```python
from build123d import *

# Parameters (mm, degrees)
SKETCH_1_W                = 1840
SKETCH_1_H                = 120
EXTRUDE_1_DEPTH           = 14
HOLE_WIZARD_1_D           = 6.6
HOLE_WIZARD_1_CBORE_D     = 11
HOLE_WIZARD_1_CBORE_DEPTH = 6.8
HOLE_WIZARD_M5_1_D        = 4.2
PATTERN_LINEAR_1_COUNT    = 27
PATTERN_LINEAR_1_PITCH    = 60
HOLE_WIZARD_12_5_12_5_2_D = 12.5
SKETCH_8_R                = 15
CUT_EXTRUDE_1_DEPTH       = 923.060735527
HOLE_WIZARD_M6_1_D        = 5
PATTERN_LINEAR_2_COUNT    = 4
PATTERN_LINEAR_2_PITCH    = 510
HOLE_WIZARD_8_5_8_5_1_D   = 8.5
SKETCH_13_R               = 42.5
CUT_EXTRUDE_2_DEPTH       = 3


with BuildPart() as part:
    # 草图1 → 凸台-拉伸1 (new body)
    with BuildSketch(Plane(origin=(0, 0, 0), x_dir=(0, 0, -1), z_dir=(1, 0, 0))):
        Rectangle(SKETCH_1_W, SKETCH_1_H)
    extrude(amount=EXTRUDE_1_DEPTH)

    # 打孔尺寸(%根据)内六角圆柱头螺钉的类型1 (through all)
    with Locations(Plane(origin=(0, 0, 0), x_dir=(0, 0, -1), z_dir=(-1, 0, 0))):
        with Locations((-896.162950904, -16.162950904), (-843.837049096, -16.162950904), (-896.162950904, 36.162950904), (-843.837049096, 36.162950904)):
            CounterBoreHole(HOLE_WIZARD_1_D / 2, HOLE_WIZARD_1_CBORE_D / 2, HOLE_WIZARD_1_CBORE_DEPTH)

    # M5 螺纹孔1 (through all)
    with Locations(Plane(origin=(14, 0, 0), x_dir=(0, 0, -1), z_dir=(1, 0, 0))):
        with Locations((-775, 26)):
            hole_wizard_m5_1 = Hole(HOLE_WIZARD_M5_1_D / 2)

    # 阵列(线性)1: M5 螺纹孔1 ×27
    with Locations(*[(0, 0, -i * PATTERN_LINEAR_1_PITCH) for i in range(1, PATTERN_LINEAR_1_COUNT)]):
        add(hole_wizard_m5_1, mode=Mode.SUBTRACT)

    # Ø12.5 (12.5) 直径孔2 (through all)
    with Locations(Plane(origin=(14, 0, 0), x_dir=(0, 0, -1), z_dir=(1, 0, 0))):
        with Locations((845, 25), (895, 25), (845, -25), (895, -25)):
            Hole(HOLE_WIZARD_12_5_12_5_2_D / 2)

    # 草图8 → 切除-拉伸1 (cut, through all)
    with BuildSketch(Plane(origin=(14, 0, 0), x_dir=(0, 0, -1), z_dir=(1, 0, 0))):
        with Locations((-870, -10)):
            Circle(SKETCH_8_R)
    extrude(amount=-CUT_EXTRUDE_1_DEPTH, mode=Mode.SUBTRACT)

    # M6 螺纹孔1 (through all)
    with Locations(Plane.ZY):
        with Locations((780, -40)):
            hole_wizard_m6_1 = Hole(HOLE_WIZARD_M6_1_D / 2)

    # 阵列(线性)2: M6 螺纹孔1 ×4
    with Locations(*[(0, 0, -i * PATTERN_LINEAR_2_PITCH) for i in range(1, PATTERN_LINEAR_2_COUNT)]):
        add(hole_wizard_m6_1, mode=Mode.SUBTRACT)

    # Ø8.5 (8.5) 直径孔1 (through all)
    with Locations(Plane(origin=(14, 0, 0), x_dir=(0, 0, -1), z_dir=(1, 0, 0))):
        with Locations((-910, 50), (-830, 50), (-910, -50), (-830, -50)):
            Hole(HOLE_WIZARD_8_5_8_5_1_D / 2)

    # 草图13 → 切除-拉伸2 (cut)
    with BuildSketch(Plane(origin=(14, 0, 0), x_dir=(0, 0, -1), z_dir=(1, 0, 0))):
        with Locations((-870, -10)):
            Circle(SKETCH_13_R)
    extrude(amount=-CUT_EXTRUDE_2_DEPTH, mode=Mode.SUBTRACT)


solid = part.part
```
For this review, take the finished solid that the model builds, in its own axes (mm). A direction names the side the tool comes from. Round coordinates to 2 decimals unless told otherwise and drop trailing zeros.
(1) Tool access review of faces 1 (the flat face through (14, 1, 13)), 2 (the flat face through (11, -9, 852)): name each direction out of +Z, -Z, +X, -X, +Y, -Y from which nothing blocks a thin tool from reaching the whole face with its end or side.
Returned:
face 1: +Z, -Z, +X, +Y, -Y
face 2: +X
(2) Wall thickness on line 1 along Z through (x, y) = (3.5, -36); line 2 along Y through (x, z) = (8.75, 295); line 3 along Z through (x, y) = (8.5, -47.5): over which ranges is each line inside the solid? List them lowest first.
Returned:
line 1: z = -920 to 838.34, 849.33 to 890.67, 901.66 to 920
line 2: y = -60 to 23.9, 28.1 to 60
line 3: z = -920 to 826.56, 833.44 to 906.56, 913.44 to 920
(3) Clearance check with flat-ended pins moving along their axes: P1, Ø3.5, axis at y = 26, z = -545, coming from the +X side; P2, Ø10.5, axis at y = -36.16, z = 843.84, coming from the -X side; P3, Ø6.5, axis at y = 26, z = -65, coming from the -X side. State where each tip first meets the part, or that it passes through.
Returned:
P1: passes through
P2: stops at x = 6.8
P3: stops at x = 0
